from build123d import *

# Parameters (mm, degrees)
SKETCH1_W           = 50
SKETCH1_H           = 150
BOSS_EXTRUDE1_DEPTH = 4
M5_TAPPED_HOLE1_D   = 4.2


with BuildPart() as part:
    # Sketch1 → Boss-Extrude1 (new, symmetric)
    with BuildSketch(Plane.XY):
        Rectangle(SKETCH1_W, SKETCH1_H)
    extrude(amount=BOSS_EXTRUDE1_DEPTH, both=True)

    # M5 Tapped Hole1 (through all)
    with Locations(Plane.XY.offset(4)):
        with Locations((-5, 60), (-5, -60), (-5, 0)):
            Hole(M5_TAPPED_HOLE1_D / 2)


solid = part.part
Build history of the part. All positions in model axes, mm. Round coordinates to 2 decimals unless told otherwise and drop trailing zeros. Write each loop counter-clockwise with the first axis right and the second up, starting at its lowest first coordinate (ties: lowest second). Pieces come first, ordered by that corner, then holes. Notation, with made-up numbers: (63.5, 40.5) - (72.5, 40.5) arc R7 ccw to (72.5, 49.5) - close; hole circle Ø2 at (58.5, -33.5). An arc over 180 degrees is marked (long way). Use CSV: the item, a comma, the result in double quotes.
(1) Pin check, flat tip, straight feed: P1, Ø5, axis at x = -5, y = -60, coming from the -Z side. Stop position of the tip, or through.
Response:
P1,"z = -4"
(2) Band-saw the part on A-A (y = 0). Write the cut outline in (x, z).
Response:
outline,"(-25, -4) - (-7.1, -4) - (-7.1, 4) - (-25, 4) - close; (-2.9, -4) - (25, -4) - (25, 4) - (-2.9, 4) - close"
(3) Band-saw the part on B-B (x = -5). Write the cut outline in (y, z).
Response:
outline,"(-75, -4) - (-62.1, -4) - (-62.1, 4) - (-75, 4) - close; (-57.9, -4) - (-2.1, -4) - (-2.1, 4) - (-57.9, 4) - close; (2.1, -4) - (57.9, -4) - (57.9, 4) - (2.1, 4) - close; (62.1, -4) - (75, -4) - (75, 4) - (62.1, 4) - close"
(4) Wall check: line 1 (Y direction, x = -4.5, z = -3). Give the ranges that are in metal, low to high.
Response:
line 1,"-75 to -62.04, -57.96 to -2.04, 2.04 to 57.96, 62.04 to 75"
(5) Mould opens along Y. For faces 1 (the cylindrical face through (-4.54, 57.95, -0.06)), 2 (the flat face through (0, -75, 0)), 3 (the flat face through (0, 1, 4)) say: pulls with the +Y half, pulls with the -Y half, needs draft (parallel to the pull), parting line crosses it, or undercut.
Response:
face 1,"undercut"
face 2,"pulls with the -Y half"
face 3,"needs draft"
